Source: three-view drawing plus pictorial views. Frame: mm from the lowest corner of the part. A direction names the side the tool comes from. Give positions to 0.01 mm unless a question says otherwise; leave off trailing zeros. Write each loop counter-clockwise with the first axis right and the second up, starting at its lowest first coordinate (ties: lowest second). Pieces come first, ordered by that corner, then holes. Notation, with made-up numbers: M -36.75,-6.75 L 6.25,-6.75 A14 cw 6.25,10.25 Z; hole C -29,60 d1. An arc over 180 degrees is marked long. Return JSON: item names as keys, results as strings.
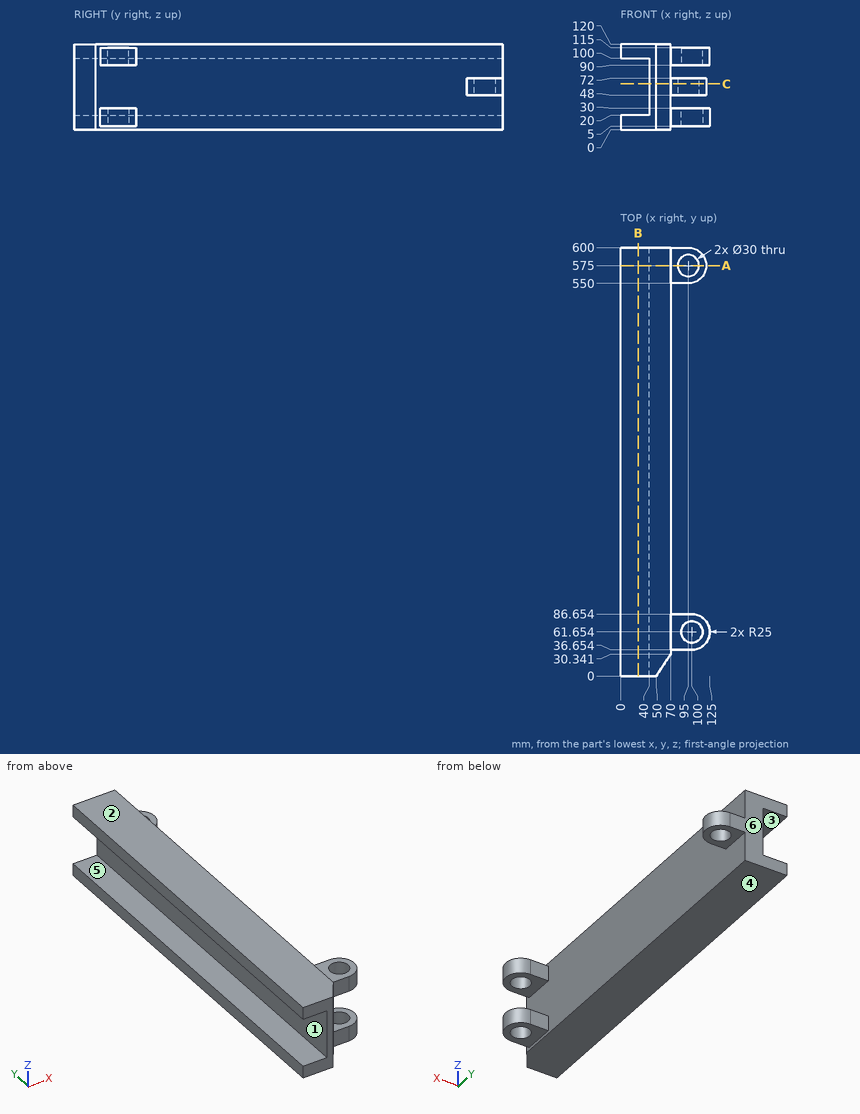
1) Set-up query: the marked faces 5 and 6. Return all of +Z, -Z, +X, -X, +Y, -Y with unobstructed straight access to the full face (end or side cutting, diameter ignored); none if empty.
Numbers:
{"face 5": "-X, +Y, -Y", "face 6": "+Z, -Z, +X, -X, +Y"}
2) Draft query along Z for the marked faces 1, 2, 3 and 4. Return one class per face: released by +Z, released by -Z, zero draft, split by the parting line, or undercut.
Numbers:
{"face 1": "undercut", "face 2": "released by +Z", "face 3": "undercut", "face 4": "released by -Z"}
3) Cut plane A-A, the plane y = 575. Return the cut outline in (x, z).
Numbers:
{"outline": "M 0,0 L 70,0 L 70,48 L 80,48 L 80,72 L 70,72 L 70,120 L 0,120 L 0,100 L 40,100 L 40,20 L 0,20 Z; M 110,48 L 120,48 L 120,72 L 110,72 Z"}
4) Line query: line 1 (Z direction, x = 19.5, y = 120); line 2 (Y direction, x = 100, z = 23.5); line 3 (Y direction, x = 95, z = 58.25). Output: solid intervals per line, ascending. Write a range as [from, to].
Numbers:
{"line 1": "z = [0, 20], [100, 120]", "line 2": "y = [36.65, 46.65], [76.65, 86.65]", "line 3": "y = [550, 560], [590, 600]"}
5) Cut plane C-C, the plane z = 64. Return the cut outline in (x, y), then the cut area to 3 significant figures.
Numbers:
{"outline": "M 40,0 L 50,0 L 70,30.34 L 70,550 L 95,550 A25 ccw 95,600 L 40,600 Z; hole C 95,575 d30", "area": "19,200 mm²"}
6) Cut plane B-B, the plane x = 24.5. Return the cut outline in (y, z), then the cut area to 3 significant figures.
Numbers:
{"outline": "M 0,0 L 600,0 L 600,20 L 0,20 Z; M 0,100 L 600,100 L 600,120 L 0,120 Z", "area": "24,000 mm²"}
7) Contact query for flat-ended pins moving along their axis: pin 1 Ø20 at (x, z) = (90, 100) entering from -Y; pin 2 Ø6 at (y, z) = (401.5, 35) entering from -X; pin 3 Ø12.5 at (x, z) = (85, 20) entering from +Y; pin 4 Ø18 at (x, y) = (95, 575) entering from -Z. Output: stop coordinate, or through.
Numbers:
{"pin 1": "stops at y = 36.65", "pin 2": "stops at x = 40", "pin 3": "stops at y = 86.65", "pin 4": "passes through"}
